Verification items for the finished model (mm, model axes). Give positions to 0.01 mm unless a question says otherwise; leave off trailing zeros. Write each loop counter-clockwise with the first axis right and the second up, starting at its lowest first coordinate (ties: lowest second). Pieces come first, ordered by that corner, then holes. Notation, with made-up numbers: (50, 78.5) -> (66, 78.5) arc R29 ccw to (66, 98.5) -> close; hole circle Ø9 at (25.25, -24.75). An arc over 180 degrees is marked (long way). Use CSV: the item, a comma, the result in double quotes. Start each with the question number.
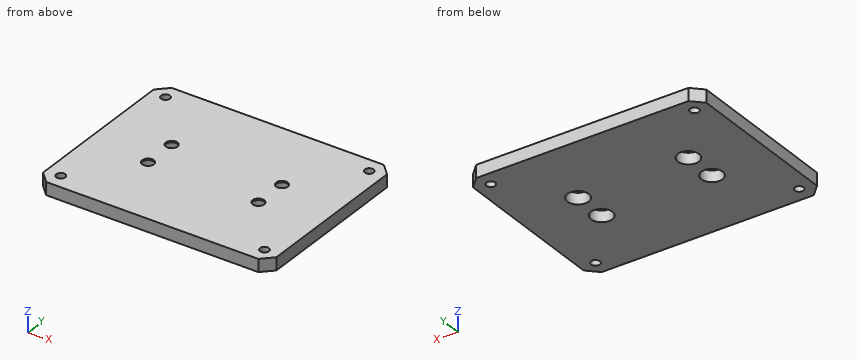
```python
from build123d import *

# Parameters (mm, degrees)
SKETCH_1_W                = 110
SKETCH_1_H                = 85
EXTRUDE_1_DEPTH           = 6
CHAMFER_1_SIZE            = 5
HOLE_WIZARD_1_D           = 5.5
HOLE_WIZARD_1_CBORE_D     = 10
HOLE_WIZARD_1_CBORE_DEPTH = 5.3
HOLE_WIZARD_M5_1_D        = 4.2
HOLE_WIZARD_M5_1_DEPTH    = 12.4
HOLE_WIZARD_M5_1_TIP      = 1.2618073


with BuildPart() as part:
    # 草图1 → 凸台-拉伸1 (new body)
    with BuildSketch(Plane.XY):
        with Locations((-21.033643231, -11.115148183)):
            Rectangle(SKETCH_1_W, SKETCH_1_H)
    extrude(amount=EXTRUDE_1_DEPTH)

    # 倒角1
    chamfer_1_edges = [part.edges().sort_by_distance(p)[0] for p in [
        (-76.033643231, 31.384851817, 3),
        (33.966356769, 31.384851817, 3),
        (33.966356769, -53.615148183, 3),
        (-76.033643231, -53.615148183, 3),
    ]]
    chamfer(chamfer_1_edges, length=CHAMFER_1_SIZE)

    # 打孔尺寸根据内六角圆柱头螺钉的类型1 (through all)
    with Locations(Plane(origin=(0, 0, 0), x_dir=(-1, 0, 0), z_dir=(0, 0, -1))):
        with Locations((47.033643231, -19.115148183), (-4.966356769, -19.115148183), (-4.966356769, -3.115148183), (47.033643231, -3.115148183)):
            CounterBoreHole(HOLE_WIZARD_1_D / 2, HOLE_WIZARD_1_CBORE_D / 2, HOLE_WIZARD_1_CBORE_DEPTH)

    # M5 螺纹孔1
    with Locations(Plane.XY.offset(6)):
        with Locations((-69.033643231, 24.384851817), (26.966356769, 24.384851817), (26.966356769, -46.615148183), (-69.033643231, -46.615148183)):
            Hole(HOLE_WIZARD_M5_1_D / 2, depth=HOLE_WIZARD_M5_1_DEPTH)
            with Locations((0, 0, -(HOLE_WIZARD_M5_1_DEPTH + HOLE_WIZARD_M5_1_TIP / 2))):  # 118° drill point
                Cone(0, HOLE_WIZARD_M5_1_D / 2, HOLE_WIZARD_M5_1_TIP, mode=Mode.SUBTRACT)


solid = part.part
```
(1) Section check B-B on z = 4.2. Give the number of separate pieces and of enclosed holes in the cut face, then the cut area to 3 significant figures.
(2) Thickness scan on line 1 (X direction, y = -3.5, z = 4.65); line 2 (Y direction, x = -43, z = 2.7); line 3 (X direction, y = 25, z = 5). Record the ranges inside material, lowest first. Write a range as from..to.
(3) Go/stop test with flat-tipped pins: pin 1 (3.5 mm diameter, centred on x = 4.97, y = -3.12, fed in from +Z); pin 2 (5 mm diameter, centred on x = -45, y = -18.5, fed in from -Z). Record where each tip stops, or that it passes through.
(4) Section check A-A on x = -47. Record the cut outline in (y, z).
Data:
1,separate pieces,"1"
1,enclosed holes,"8"
1,area,"8,930 mm2"
2,line 1,"x = -76.03..-52.02, -42.05..-0.02, 9.95..33.97"
2,line 2,"y = -53.62..-22.07, -16.16..-6.07, -0.16..31.38"
2,line 3,"x = -76.03..-71.04, -67.03..24.96, 28.97..33.97"
3,pin 1,"passes through"
3,pin 2,"stops at z = 5.3"
4,outline,"(-53.62, 0) -> (-24.12, 0) -> (-24.12, 5.3) -> (-21.86, 5.3) -> (-21.86, 6) -> (-53.62, 6) -> close; (-16.37, 5.3) -> (-14.12, 5.3) -> (-14.12, 0) -> (-8.12, 0) -> (-8.12, 5.3) -> (-5.86, 5.3) -> (-5.86, 6) -> (-16.37, 6) -> close; (-0.37, 5.3) -> (1.88, 5.3) -> (1.88, 0) -> (31.38, 0) -> (31.38, 6) -> (-0.37, 6) -> close"
